Geometry check sheet. Reference: the model listing, model coordinates, mm. A direction names the side the tool comes from. Give positions to 0.01 mm unless a question says otherwise; leave off trailing zeros. Loops run counter-clockwise (first coordinate to the right, second up) from the corner with the lowest first, then second, coordinate; pieces in that order, holes last. Notation, with made-up numbers: (-38.5, -21) -> (7.5, -21) arc R16 cw to (7.5, -16) -> close; hole circle Ø11 at (-14.75, 4.5). An arc over 180 degrees is marked (long way). One line per question, with ' | ' between items.
from build123d import *

# Parameters (mm, degrees)
EXTRUDE_1_DEPTH     = 20
SKETCH_2_R          = 4.5
CUT_EXTRUDE_1_DEPTH = 5
SKETCH_3_R          = 2.8
CUT_EXTRUDE_2_DEPTH = 31.886890423


with BuildPart() as part:
    # 草图1 → 拉伸1 (new body)
    with BuildSketch(Plane(origin=(0, 0, 0), x_dir=(1, 0, 0), z_dir=(0, 1, 0))):
        Polygon((0, 0), (18.5, 0), (23, 9), (0, 9), align=None)
    extrude(amount=EXTRUDE_1_DEPTH)

    # 草图2 → 切除-拉伸1 (cut)
    with BuildSketch(Plane(origin=(0, 0, -9), x_dir=(-1, 0, 0), z_dir=(0, 0, -1))):
        with Locations((-8, 10)):
            Circle(SKETCH_2_R)
    extrude(amount=-CUT_EXTRUDE_1_DEPTH, mode=Mode.SUBTRACT)

    # 草图3 → 切除-拉伸2 (cut, through all)
    with BuildSketch(Plane(origin=(0, 0, -4), x_dir=(-1, 0, 0), z_dir=(0, 0, -1))):
        with Locations((-8, 10)):
            Circle(SKETCH_3_R)
    extrude(amount=-CUT_EXTRUDE_2_DEPTH, mode=Mode.SUBTRACT)


solid = part.part
Item 1: Sectioned sample at C-C (z = -2). Record the cut outline in (x, y).
Result:
outline: (0, 0) -> (19.5, 0) -> (19.5, 20) -> (0, 20) -> close; hole circle Ø5.6 at (8, 10)
Item 2: Depth check by flat-ended pin: pin 1 Ø1 at (x, z) = (16, -1) entering from -Y; pin 2 Ø5 at (y, z) = (16.5, -2.5) entering from +X; pin 3 Ø5 at (x, y) = (8, 10) entering from +Z. Enter the tip coordinate at first touch or a pass-through.
Result:
pin 1: y = 0 | pin 2: x = 21 | pin 3: through
Item 3: Set-up check for faces 1 (the face through (14, 10, -9)), 2 (the face through (3.708, 11.352, -6.535)): record each of +Z, -Z, +X, -X, +Y, -Y from which the full face is reachable in a straight line by a thin tool's end or side.
Result:
face 1: -Z, +X, -X, +Y, -Y | face 2: -Z
Item 4: Sectioned sample at A-A (y = 10). Record the cut outline in (x, z).
Result:
outline: (0, -9) -> (3.5, -9) -> (3.5, -4) -> (5.2, -4) -> (5.2, 0) -> (0, 0) -> close; (10.8, -4) -> (12.5, -4) -> (12.5, -9) -> (23, -9) -> (18.5, 0) -> (10.8, 0) -> close
Item 5: Sectioned sample at B-B (x = 9.25). Record the cut outline in (y, z), plus the area to 3 significant figures.
Result:
outline: (0, -9) -> (5.68, -9) -> (5.68, -4) -> (7.49, -4) -> (7.49, 0) -> (0, 0) -> close; (12.51, -4) -> (14.32, -4) -> (14.32, -9) -> (20, -9) -> (20, 0) -> (12.51, 0) -> close | area: 117 mm2
Item 6: Scan lines: probe 1 along Y at (x, z) = (8, -2.95); probe 2 along Y at (x, z) = (8, -6.4); probe 3 along X at (y, z) = (8, -6.5). Record each from-to range of solid material in increasing order.
Result:
probe 1: 0 to 7.2, 12.8 to 20 | probe 2: 0 to 5.5, 14.5 to 20 | probe 3: 0 to 3.97, 12.03 to 21.75
Item 7: Release check for a two-part mould opening along X. For faces 3 (the face through (20.7, 9.9, -4.4)), 4 (the face through (8, 7, -4)), 5 (the face through (11, 10, 0)) record: pulls with the +X half, pulls with the -X half, needs draft (parallel to the pull), parting line crosses it, or undercut.
Result:
face 3: pulls with the +X half | face 4: undercut | face 5: needs draft
Item 8: Sectioned sample at D-D (z = -0.5). Record the cut outline in (x, y).
Result:
outline: (0, 0) -> (18.75, 0) -> (18.75, 20) -> (0, 20) -> close; hole circle Ø5.6 at (8, 10)
